Read the model definition and answer for the solid it produces. Units are mm, in the model's axes. Face numbers are marked on the shaded views. Coordinates: 2 decimals unless noted, no trailing zeros. Loops run counter-clockwise (first coordinate to the right, second up) from the corner with the lowest first, then second, coordinate; pieces in that order, holes last. Notation, with made-up numbers: (-28.75, -26) -> (-12.75, -26) arc R5 ccw to (-12.75, -17) -> close; hole circle Ø4 at (12.25, 10.25). An arc over 180 degrees is marked (long way). Answer as CSV lines item,"result".
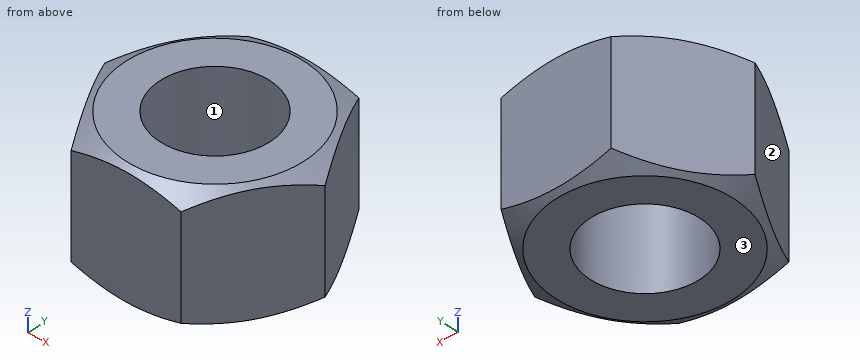
```python
from build123d import *

# Parameters (mm, degrees)
BOSS_EXTRUDE1_DEPTH = 15.8
SKETCH3_R           = 6.92
CUT_EXTRUDE1_DEPTH  = 25.2


with BuildPart() as part:
    # Sketch1 → Boss-Extrude1 (new body)
    with BuildSketch(Plane.XY):
        Polygon((13.856406461, 0), (6.92820323, 12), (-6.92820323, 12), (-13.856406461, 0), (-6.92820323, -12), (6.92820323, -12), align=None)
    extrude(amount=BOSS_EXTRUDE1_DEPTH)

    # Sketch2 → Cut-Revolve1 (revolve, cut)
    with BuildSketch(Plane(origin=(0, 0, 0), x_dir=(1, 0, 0), z_dir=(0, 1, 0))):
        Polygon((13.856406461, -1.5), (6.92820323, 2.5), (16.856406461, 3.696152423), align=None)
        Polygon((13.856406461, -14.3), (6.92820323, -18.3), (16.856406461, -19.496152423), align=None)
    revolve(axis=Axis((0, 0, 0), (0, 0, 1)), mode=Mode.SUBTRACT)

    # Sketch3 → Cut-Extrude1 (cut, through all)
    with BuildSketch(Plane.XY):
        Circle(SKETCH3_R)
    extrude(amount=CUT_EXTRUDE1_DEPTH, mode=Mode.SUBTRACT)


solid = part.part
```
Q1. For a pull along X with two mould halves and no side action, classify the marked faces 1, 2 and 3 as pulls with the +X half, pulls with the -X half, needs draft (parallel to the pull), parting line crosses it, or undercut.
Results:
face 1,"undercut"
face 2,"pulls with the -X half"
face 3,"needs draft"
Q2. A cutting plane is placed at B-B, the plane z = 13.25. Write down the section's boundary in (x, y).
Results:
outline,"(-13.86, 0) -> (-6.93, -12) -> (6.93, -12) -> (13.86, 0) -> (6.93, 12) -> (-6.93, 12) -> close; hole circle Ø13.84 at (0, 0)"
Q3. A cutting plane is placed at A-A, the plane x = 0. Write down the section's boundary in (y, z), and give its area (3 significant figures).
Results:
outline,"(-12, 0.43) -> (-11.26, 0) -> (-6.92, 0) -> (-6.92, 15.8) -> (-11.26, 15.8) -> (-12, 15.37) -> close; (6.92, 0) -> (11.26, 0) -> (12, 0.43) -> (12, 15.37) -> (11.26, 15.8) -> (6.92, 15.8) -> close"
area,"160 mm²"
Q4. Find the intervals of material crossed by probe 1 along Y at (x, z) = (0, 6.5); probe 2 along X at (y, z) = (-1.25, 5.75); probe 3 along Y at (x, z) = (-5, 11.75), in increasing order. Write a range as [from, to].
Results:
probe 1,"y = [-12, -6.92], [6.92, 12]"
probe 2,"x = [-13.13, -6.81], [6.81, 13.13]"
probe 3,"y = [-12, -4.78], [4.78, 12]"
Q5. Given pin 1 Ø8 at (y, z) = (-9, 6.5) entering from -X; pin 2 Ø5 at (y, z) = (-1, 10.5) entering from +X, each flat-ended and moving along its own axis, determine where each tip first touches the part or whether it passes through.
Results:
pin 1,"stops at x = -10.97"
pin 2,"stops at x = 13.86"
